Here's how the part is built. I have some questions about the finished solid (model axes, mm). Round coordinates to 2 decimals unless told otherwise and drop trailing zeros. Order: outer loops, then holes, each group sorted by start corner. A loop starts at its lowest first (then second) coordinate and runs counter-clockwise, first axis right, second up. Notation, with made-up numbers: (80.25, -4) -> (139.25, -4) arc R20 cw to (139.25, 0) -> close; hole circle Ø2 at (33, -13). An arc over 180 degrees is marked (long way). One line per item, written item: value.
```python
from build123d import *

# Parameters (mm, degrees)
SKETCH1_W           = 320
SKETCH1_H           = 370
SKETCH1_R           = 50
BOSS_EXTRUDE1_DEPTH = 10


with BuildPart() as part:
    # Sketch1 → Boss-Extrude1 (new body)
    with BuildSketch(Plane.XY):
        with Locations((160, 185)):
            Rectangle(SKETCH1_W, SKETCH1_H)
        with Locations((160, 120)):
            Circle(SKETCH1_R, mode=Mode.SUBTRACT)
    extrude(amount=BOSS_EXTRUDE1_DEPTH)


solid = part.part
```
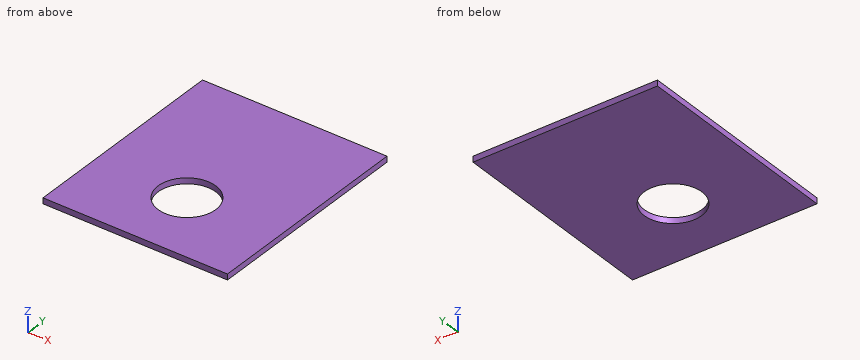
Q1. I want a section at A-A on y = 120. Write out the boundary of the cut face in (x, z).
Answers:
outline: (0, 0) -> (110, 0) -> (110, 10) -> (0, 10) -> close; (210, 0) -> (320, 0) -> (320, 10) -> (210, 10) -> close
Q2. I want a section at B-B on x = 160. Write out the boundary of the cut face in (y, z).
Answers:
outline: (0, 0) -> (70, 0) -> (70, 10) -> (0, 10) -> close; (170, 0) -> (370, 0) -> (370, 10) -> (170, 10) -> close
Q3. I want a section at C-C on z = 6.25. Write out the boundary of the cut face in (x, y), then the cut area to 3 significant figures.
Answers:
outline: (0, 0) -> (320, 0) -> (320, 370) -> (0, 370) -> close; hole circle Ø100 at (160, 120)
area: 111,000 mm2
Q4. I need wall thicknesses on line 1 along Y through (x, z) = (160, 3.25); line 2 along Y through (x, z) = (136, 4.25); line 3 along X through (y, z) = (107.5, 4). Which ranges of each line are inside material? Lowest first, please.
Answers:
line 1: 0 to 70, 170 to 370
line 2: 0 to 76.14, 163.86 to 370
line 3: 0 to 111.59, 208.41 to 320
